from build123d import *

# Parameters (mm, degrees)
SKETCH_1_W      = 30
SKETCH_1_H      = 30
SKETCH_1_W_2    = 26
SKETCH_1_H_2    = 26
EXTRUDE_1_DEPTH = 556


with BuildPart() as part:
    # 草图1 → 凸台-拉伸1 (new, symmetric)
    with BuildSketch(Plane.XY):
        Rectangle(SKETCH_1_W, SKETCH_1_H)
        Rectangle(SKETCH_1_W_2, SKETCH_1_H_2, mode=Mode.SUBTRACT)
    extrude(amount=EXTRUDE_1_DEPTH, both=True)


solid = part.part
Could you check a few things on this model? Use its own coordinates, in mm. A direction names the side the tool comes from. Round coordinates to 2 decimals unless told otherwise and drop trailing zeros. Order: outer loops, then holes, each group sorted by start corner. A loop starts at its lowest first (then second) coordinate and runs counter-clockwise, first axis right, second up.
(1) Which directions (+Z, -Z, +X, -X, +Y, -Y) give clear straight access to the entire face, cutting with the end or side of a thin tool? Please do faces 1 (the flat face through (13, 0, 8)), 2 (the flat face through (-14, 0, -556)).
Response values:
face 1: +Z, -Z
face 2: -Z, +X, -X, +Y, -Y
(2) Imagine slicing it at C-C (z = 258.5). Write out the boundary of the cut face in (x, y), plus the area to 3 significant figures.
Response values:
outline: (-15, -15) - (15, -15) - (15, 15) - (-15, 15) - close; hole (-13, -13) - (13, -13) - (13, 13) - (-13, 13) - close
area: 224 mm2
(3) Imagine slicing it at A-A (x = -8.5). Write out the boundary of the cut face in (y, z).
Response values:
outline: (-15, -556) - (-13, -556) - (-13, 556) - (-15, 556) - close; (13, -556) - (15, -556) - (15, 556) - (13, 556) - close
(4) Please list where this line runs through material, in increasing order: line 1 along Y through (x, z) = (5, 12.5).
Response values:
line 1: y = -15 to -13, 13 to 15
(5) If we mould it in two halves opening along Y, with no side actions, what happens to faces 3 (the flat face through (0, -15, 8)), 4 (the flat face through (0, 13, 8)), 5 (the flat face through (15, 0, 8))? For each: released by +Y, released by -Y, zero draft, split by the parting line, or undercut.
Response values:
face 3: released by -Y
face 4: undercut
face 5: zero draft
